```python
from build123d import *

# Parameters (mm, degrees)
SKETCH1_W             = 25
SKETCH1_H             = 23
BOSS_EXTRUDE1_DEPTH   = 10
SKETCH2_R             = 6.05
CUT_EXTRUDE1_DEPTH    = 20.710403344
CHAMFER1_SIZE         = 2
M4_TAPPED_HOLE1_D     = 3.3
M4_TAPPED_HOLE1_DEPTH = 10.1
M4_TAPPED_HOLE1_TIP   = 0.991420021


with BuildPart() as part:
    # Sketch1 → Boss-Extrude1 (new body)
    with BuildSketch(Plane.XY):
        Rectangle(SKETCH1_W, SKETCH1_H)
    extrude(amount=BOSS_EXTRUDE1_DEPTH)

    # Sketch2 → Cut-Extrude1 (cut, through all)
    with BuildSketch(Plane.XY.offset(10)):
        with Locations((0, 3.5)):
            Circle(SKETCH2_R)
    extrude(amount=-CUT_EXTRUDE1_DEPTH, mode=Mode.SUBTRACT)

    # Chamfer1
    chamfer1_edges = [part.edges().sort_by_distance(p)[0] for p in [
        (-12.5, 11.5, 5),
        (12.5, 11.5, 5),
    ]]
    chamfer(chamfer1_edges, length=CHAMFER1_SIZE)

    # M4 Tapped Hole1
    with Locations(Plane.XZ.offset(11.5)):
        with Locations((-7, 5), (7, 5)):
            Hole(M4_TAPPED_HOLE1_D / 2, depth=M4_TAPPED_HOLE1_DEPTH)
            with Locations((0, 0, -(M4_TAPPED_HOLE1_DEPTH + M4_TAPPED_HOLE1_TIP / 2))):  # 118° drill point
                Cone(0, M4_TAPPED_HOLE1_D / 2, M4_TAPPED_HOLE1_TIP, mode=Mode.SUBTRACT)

    # Sketch5 → M4 Tapped Hole2 (revolve, cut)
    with BuildSketch(Plane(origin=(-12.5, 3.5, 5), x_dir=(0, 0, 1), z_dir=(0, 1, 0))):
        Polygon((0, 0), (0, 11.091420021), (1.65, 10.1), (1.65, 0), align=None)
    m4_tapped_hole2 = revolve(axis=Axis((-18.85, 3.5, 5), (1, 0, 0)), mode=Mode.SUBTRACT)

    # Mirror1: M4 Tapped Hole2 across plane
    add(m4_tapped_hole2.mirror(Plane(origin=(0, 0, 0), x_dir=(0, 0, 1), z_dir=(1, 0, 0))), mode=Mode.SUBTRACT)


solid = part.part
```
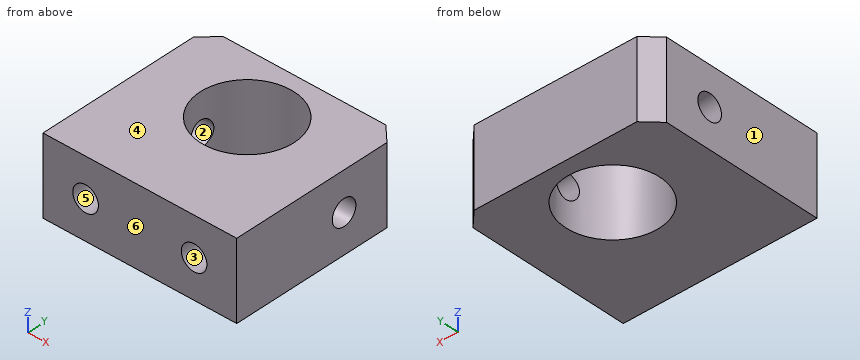
CAD build for the part. Positions are in the model's coordinates, mm. Face numbers are marked on the shaded views. A direction names the side the tool comes from. Round coordinates to 2 decimals unless told otherwise and drop trailing zeros. Loops run counter-clockwise (first coordinate to the right, second up) from the corner with the lowest first, then second, coordinate; pieces in that order, holes last. Notation, with made-up numbers: M 14.5,71 L 30.5,71 A24 cw 30.5,95 Z; hole C 11.25,37.25 d7. An arc over 180 degrees is marked long. Use a Markdown table: item, result. Add a question column.
(1) Cut at B-B (z = 8). Give the cut face in (x, y), and give its area (3 significant figures).
(2) Drill centre lines: line 1 (X direction, y = -8.5, z = 5); line 2 (Z direction, x = 11.25, y = 3.5); line 3 (Y direction, x = -11.5, z = 5). Where is each one in solid material? Low to high.
(3) Which spindle directions (+Z, -Z, +X, -X, +Y, -Y) get a long thin tool onto all of the face, cutting with end or side? Do the marked faces 5 and 6. Say none if no direction does.
(4) Flat gauge pins, fed straight in: pin 1 (7.5 mm diameter, centred on x = 0, y = 3.5, fed in from -Z); pin 2 (4.5 mm diameter, centred on x = -7, z = 5, fed in from -Y). Where does each tip first touch, or does it go through?
(5) Cut at A-A (x = 0). Give the cut face in (y, z), and give its area (3 significant figures).
(6) Pull direction Z, two halves, no side cores. Call the marked faces 1, 2, 3 and 4: +Z half, -Z half, draft (parallel to the pull), parting line (faces both ways), or undercut.
(7) Cut at C-C (y = 1.25). Give the cut face in (x, z), and give its area (3 significant figures).
Geometry says:
| question | item | result |
|---|---|---|
| 1 | outline | M -12.5,-11.5 L 12.5,-11.5 L 12.5,9.5 L 10.5,11.5 L -10.5,11.5 L -12.5,9.5 Z; hole C 0,3.5 d12.1 |
| 1 | area | 456 mm² |
| 2 | line 1 | x = -12.5 to -8.65, -5.35 to 5.35, 8.65 to 12.5 |
| 2 | line 2 | z = 0 to 3.35, 6.65 to 10 |
| 2 | line 3 | y = -11.5 to 1.85, 5.15 to 10.5 |
| 3 | face 5 | -Y |
| 3 | face 6 | +Z, -Z, +X, -X, -Y |
| 4 | pin 1 | passes through |
| 4 | pin 2 | stops at y = -11.5 |
| 5 | outline | M -11.5,0 L -2.55,0 L -2.55,10 L -11.5,10 Z; M 9.55,0 L 11.5,0 L 11.5,10 L 9.55,10 Z |
| 5 | area | 109 mm² |
| 6 | face 1 | draft |
| 6 | face 2 | undercut |
| 6 | face 3 | undercut |
| 6 | face 4 | +Z half |
| 7 | outline | M -12.5,0 L -5.62,0 L -5.62,10 L -12.5,10 Z; M 5.62,0 L 12.5,0 L 12.5,10 L 5.62,10 Z |
| 7 | area | 138 mm² |
